Source: CAD feature listing. Evaluate the final solid. Frame: model axes, mm. Face numbers are marked on the shaded views. Give positions to 0.01 mm unless a question says otherwise; leave off trailing zeros. Loops run counter-clockwise (first coordinate to the right, second up) from the corner with the lowest first, then second, coordinate; pieces in that order, holes last. Notation, with made-up numbers: M 85.5,23.5 L 111.5,23.5 A19 cw 111.5,35.5 Z; hole C 70.25,-22.5 d3. An arc over 180 degrees is marked long. Put each result on its own line as item: value.
from build123d import *

# Parameters (mm, degrees)
SKETCH_1_W      = 64
SKETCH_1_H      = 38
SKETCH_1_W_2    = 60.4
SKETCH_1_H_2    = 34.4
EXTRUDE_1_DEPTH = 2.5


with BuildPart() as part:
    # 草图1 → 凸台-拉伸1 (new, symmetric)
    with BuildSketch(Plane.XY):
        Rectangle(SKETCH_1_W, SKETCH_1_H)
        Rectangle(SKETCH_1_W_2, SKETCH_1_H_2, mode=Mode.SUBTRACT)
    extrude(amount=EXTRUDE_1_DEPTH, both=True)


solid = part.part
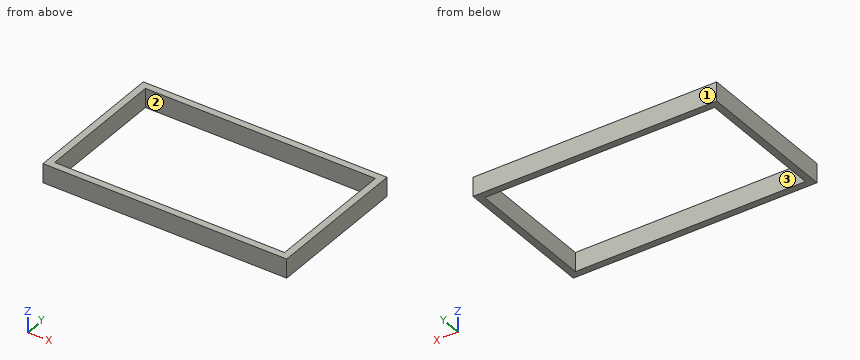
1. Draft query along X for the marked faces 1, 2 and 3. Return one class per face: pulls with the +X half, pulls with the -X half, needs draft (parallel to the pull), parting line crosses it, or undercut.
Found:
face 1: needs draft
face 2: undercut
face 3: undercut
2. Section query A-A (x = 24.5). Output: boundary loops of the cut face in (y, z), plus the area to 3 significant figures.
Found:
outline: M -19,-2.5 L -17.2,-2.5 L -17.2,2.5 L -19,2.5 Z; M 17.2,-2.5 L 19,-2.5 L 19,2.5 L 17.2,2.5 Z
area: 18.0 mm^2
3. Section query B-B (y = 2). Output: boundary loops of the cut face in (x, z), plus the area to 3 significant figures.
Found:
outline: M -32,-2.5 L -30.2,-2.5 L -30.2,2.5 L -32,2.5 Z; M 30.2,-2.5 L 32,-2.5 L 32,2.5 L 30.2,2.5 Z
area: 18.0 mm^2
4. Section query C-C (z = -1.7). Output: boundary loops of the cut face in (x, y), plus the area to 3 significant figures.
Found:
outline: M -32,-19 L 32,-19 L 32,19 L -32,19 Z; hole M -30.2,-17.2 L 30.2,-17.2 L 30.2,17.2 L -30.2,17.2 Z
area: 354 mm^2
5. Material intervals for line 1 (Y direction, x = 12, z = 0.6); line 2 (X direction, y = 12, z = -0.6), sorted ascending. Write a range as from..to.
Found:
line 1: -19..-17.2, 17.2..19
line 2: -32..-30.2, 30.2..32
